CAD build for the part. Positions are in the model's coordinates, mm. A direction names the side the tool comes from. Coordinates: 2 decimals unless noted, no trailing zeros. Loops run counter-clockwise (first coordinate to the right, second up) from the corner with the lowest first, then second, coordinate; pieces in that order, holes last. Notation, with made-up numbers: (75.5, 78) -> (125.5, 78) arc R23 ccw to (125.5, 105) -> close; hole circle Ø9 at (13.5, 40). An arc over 180 degrees is marked (long way). Write item = value, one per line. Start each with the question number.
(1) Flat gauge pins, fed straight in: P1, Ø8, axis at x = 43.5, z = 12.5, coming from the +Y side; P2, Ø5, axis at y = 15, z = 19.5, coming from the +X side. Where does each tip first touch, or does it go through?
(2) Drill centre lines: line 1 (Z direction, x = 4.5, y = 30); line 2 (Z direction, x = 48.5, y = 6); line 3 (X direction, y = 62, z = 13). Where is each one in solid material? Low to high. Write a range as from..to.
(3) Band-saw the part on B-B (x = 51.5). Write the cut outline in (y, z).
(4) Band-saw the part on A-A (y = 30). Write the cut outline in (x, z).
(5) Band-saw the part on C-C (z = 6). Write the cut outline in (x, y).
(6) Pull direction Z, two halves, no side cores. Call faces 4 (the face through (8, 21, 26)), 5 (the face through (30, 0, 0)), 6 (the face through (54, 5, -8)): +Z half, -Z half, draft (parallel to the pull), parting line (faces both ways), or undercut.
(7) Band-saw the part on D-D (z = -10.5). Write the cut outline in (x, y), and give its area (3 significant figures).
(8) Tool access for faces 1 (the face through (60, 5, -17)), 2 (the face through (54, 5, 8)), 3 (the face through (35, 10, 0)): list every direction of +Z, -Z, +X, -X, +Y, -Y with a clear straight run to the whole face (end or side of a thin tool).
```python
from build123d import *

# Parameters (mm, degrees)
L_BRACKET_BODY_DEPTH  = 26
BASE_U_SLOT_DEPTH     = 86.44588931
UPRIGHT_HOLE_SKETCH_R = 8
UPRIGHT_HOLE_16_DEPTH = 87.029064856
CHAMFER_11X45_SIZE    = 11


with BuildPart() as part:
    # L-Profile Sketch → L-Bracket Body (new, symmetric)
    with BuildSketch(Plane.XY):
        Polygon((0, 0), (0, 65), (10, 65), (10, 10), (60, 10), (60, 0), align=None)
    extrude(amount=L_BRACKET_BODY_DEPTH, both=True)

    # Base Slot Sketch → Base U-Slot (cut, through all)
    with BuildSketch(Plane(origin=(0, 10, 0), x_dir=(1, 0, 0), z_dir=(0, 1, 0))):
        with BuildLine():
            Line((48, 8), (60, 8))
            Line((60, 8), (60, -8))
            Line((60, -8), (48, -8))
            ThreePointArc((48, -8), (40, 0), (48, 8))
        make_face()
    extrude(amount=-BASE_U_SLOT_DEPTH, mode=Mode.SUBTRACT)

    # Upright Hole Sketch → Upright Hole Ø16 (cut, through all)
    with BuildSketch(Plane(origin=(10, 0, 0), x_dir=(0, 0, -1), z_dir=(1, 0, 0))):
        with Locations(Location((-6, 30, 0), (0, 0, 90))):
            Circle(UPRIGHT_HOLE_SKETCH_R)
    extrude(amount=-UPRIGHT_HOLE_16_DEPTH, mode=Mode.SUBTRACT)

    # Chamfer 11x45°
    chamfer_11x45_edges = [part.edges().sort_by_distance(p)[0] for p in [
        (5, 65, -26),
    ]]
    chamfer(chamfer_11x45_edges, length=CHAMFER_11X45_SIZE)


solid = part.part
```
Findings below:
q1.P1 = 10
q1.P2 = 10
q2.line_1 = -26..-2, 14..26
q2.line_2 = -26..-8, 8..26
q2.line_3 = 0..10
q3.outline = (0, -26) -> (10, -26) -> (10, -8) -> (0, -8) -> close; (0, 8) -> (10, 8) -> (10, 26) -> (0, 26) -> close
q4.outline = (0, -26) -> (10, -26) -> (10, -2) -> (0, -2) -> close; (0, 14) -> (10, 14) -> (10, 26) -> (0, 26) -> close
q5.outline = (0, 0) -> (42.71, 0) -> (42.71, 10) -> (10, 10) -> (10, 22) -> (0, 22) -> close; (0, 38) -> (10, 38) -> (10, 65) -> (0, 65) -> close
q6.face_4 = +Z half
q6.face_5 = draft
q6.face_6 = undercut
q7.outline = (0, 0) -> (60, 0) -> (60, 10) -> (10, 10) -> (10, 65) -> (0, 65) -> close
q7.area = 1,150 mm²
q8.face_1 = +Z, -Z, +X, +Y, -Y
q8.face_2 = +X, +Y, -Y
q8.face_3 = +Z, -Z, +X, +Y
